Could you check a few things on this model? Use its own coordinates, in mm. Coordinates: 2 decimals unless noted, no trailing zeros. Write each loop counter-clockwise with the first axis right and the second up, starting at its lowest first coordinate (ties: lowest second). Pieces come first, ordered by that corner, then holes.
Item 1: I want a section at A-A on x = -4.5. Please give me the cut outline in (y, z).
Item 2: If I drill on probe 1 along Z at (x, y) = (5, -0.5); probe 2 along Z at (x, y) = (-7, -0.25); probe 3 along Z at (x, y) = (6, -1), over which ranges is the centre line in solid material (lowest first)?
Item 3: I want a section at C-C on z = 339. Please give me the cut outline in (x, y).
Item 4: I want a section at B-B on y = 1.5. State how many separate pieces and enclosed holes the cut face has, then the cut area to 3 significant figures.
Item 5: For P1, Ø6, axis at x = 5.13, z = 242, coming from the +Y side; P2, Ø4, axis at x = 3.5, z = 241, coming from the -Y side; P3, Ø1.5, axis at y = 8, z = 372.5, coming from the +X side; P4, Ø2.5, axis at x = 4.5, z = 650.5, coming from the -Y side, each with a flat end and sliding along its axis, tell me the tip position at first contact or that it passes through.
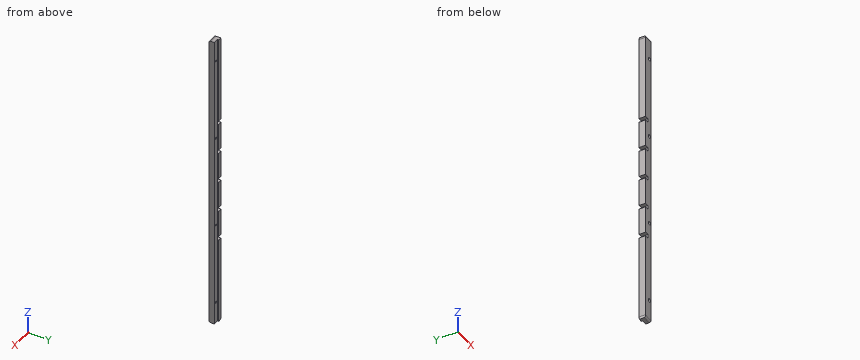
from build123d import *

# Parameters (mm, degrees)
EXTRUDE_1_DEPTH           = 700
HOLE_WIZARD_1_D           = 4.5
HOLE_WIZARD_1_CBORE_D     = 8
HOLE_WIZARD_1_CBORE_DEPTH = 4.6
SKETCH_5_W                = 9
SKETCH_5_H                = 15
CUT_EXTRUDE_1_DEPTH       = 9
CHAMFER_1_SIZE            = 5
CHAMFER_1_SIZE2           = 1
CHAMFER_2_SIZE            = 1
CHAMFER_2_SIZE2           = 5
FILLET_1_R                = 4


with BuildPart() as part:
    # 草图1 → 凸台-拉伸1 (new body)
    with BuildSketch(Plane.XY):
        Polygon((-9.367113838, -5.483188588), (11.132886162, -5.483188588), (11.132886162, 6.516811412), (-0.867113838, 6.516811412), (-0.867113838, 9.516811412), (-9.367113838, 9.516811412), align=None)
    extrude(amount=EXTRUDE_1_DEPTH)

    # 打孔尺寸根据内六角圆柱头螺钉的类型1 (through all)
    with Locations(Plane(origin=(0, -5.483188588, 0), x_dir=(-1, 0, 0), z_dir=(0, -1, 0))):
        with Locations((-5.132886162, -650), (-5.132886162, -458), (-5.132886162, -242), (-5.132886162, -50)):
            CounterBoreHole(HOLE_WIZARD_1_D / 2, HOLE_WIZARD_1_CBORE_D / 2, HOLE_WIZARD_1_CBORE_DEPTH)

    # 草图5 → 切除-拉伸1 (cut)
    with BuildSketch(Plane.ZY.offset(9.367113838)):
        with Locations((206, 2.016811412)):
            Rectangle(SKETCH_5_W, SKETCH_5_H)
        with Locations((278, 2.016811412)):
            Rectangle(SKETCH_5_W, SKETCH_5_H)
        with Locations((350, 2.016811412)):
            Rectangle(SKETCH_5_W, SKETCH_5_H)
        with Locations((422, 2.016811412)):
            Rectangle(SKETCH_5_W, SKETCH_5_H)
        with Locations((494, 2.016811412)):
            Rectangle(SKETCH_5_W, SKETCH_5_H)
    extrude(amount=-CUT_EXTRUDE_1_DEPTH, mode=Mode.SUBTRACT)

    # 倒角1
    chamfer_1_edges = [part.edges().sort_by_distance(p)[0] for p in [
        (-9.367113838, 2.016811412, 700),
    ]]
    chamfer_1_side = [part.faces().sort_by_distance(p)[0] for p in [
        (-9.367113838, 2.016811412, 599.25),
    ]]
    chamfer(chamfer_1_edges, length=CHAMFER_1_SIZE, length2=CHAMFER_1_SIZE2, reference=chamfer_1_side[0])

    # 倒角2
    chamfer_2_edges = [part.edges().sort_by_distance(p)[0] for p in [
        (-9.367113838, 2.016811412, 0),
    ]]
    chamfer_2_side = [part.faces().sort_by_distance(p)[0] for p in [
        (0.31935025, 1.221231301, 0),
    ]]
    chamfer(chamfer_2_edges, length=CHAMFER_2_SIZE, length2=CHAMFER_2_SIZE2, reference=chamfer_2_side[0])

    # 圆角1
    fillet_1_edges = [part.edges().sort_by_distance(p)[0] for p in [
        (1.382886162, -5.483188588, 700),
        (1.382886162, -5.483188588, 0),
    ]]
    fillet(fillet_1_edges, radius=FILLET_1_R)


solid = part.part
Response values:
1. outline: (-5.48, 4) arc R4 ccw to (-1.48, 0) - (9.52, 0) - (9.52, 201.5) - (-5.48, 201.5) - close; (-5.48, 210.5) - (9.52, 210.5) - (9.52, 273.5) - (-5.48, 273.5) - close; (-5.48, 282.5) - (9.52, 282.5) - (9.52, 345.5) - (-5.48, 345.5) - close; (-5.48, 354.5) - (9.52, 354.5) - (9.52, 417.5) - (-5.48, 417.5) - close; (-5.48, 426.5) - (9.52, 426.5) - (9.52, 489.5) - (-5.48, 489.5) - close; (-5.48, 498.5) - (9.52, 498.5) - (9.52, 700) - (-1.48, 700) arc R4 ccw to (-5.48, 696) - close
2. probe 1: z = 0 to 47.75, 52.25 to 239.75, 244.25 to 455.75, 460.25 to 647.75, 652.25 to 700
2. probe 2: z = 0 to 201.5, 210.5 to 273.5, 282.5 to 345.5, 354.5 to 417.5, 426.5 to 489.5, 498.5 to 700
2. probe 3: z = 0 to 46.1, 53.9 to 238.1, 245.9 to 454.1, 461.9 to 646.1, 653.9 to 700
3. outline: (-9.37, -5.48) - (11.13, -5.48) - (11.13, 6.52) - (-0.87, 6.52) - (-0.87, 9.52) - (-9.37, 9.52) - close
4. separate pieces: 1
4. enclosed holes: 4
4. area: 13,900 mm2
5. P1: stops at y = 6.52
5. P2: stops at y = -0.88
5. P3: stops at x = -0.87
5. P4: passes through
